For this review, use the dimensioned drawing (mm, ordinates from the lowest corner) and the shaded views. Coordinates: 2 decimals unless noted, no trailing zeros. Loops run counter-clockwise (first coordinate to the right, second up) from the corner with the lowest first, then second, coordinate; pieces in that order, holes last. Notation, with made-up numbers: (-8.5, -10.75) - (44.5, -10.75) arc R19 cw to (44.5, 26.25) - close; hole circle Ø4 at (33, 1). An arc over 180 degrees is marked (long way). Answer in a Markdown table with one row per item. Add a question column.
(1) For P1, Ø1.5, axis at x = 14, z = 13.5, coming from the -Y side; P2, Ø12, axis at y = 10.5, z = 23, coming from the -X side (1 decimal); P3, Ø9.5, axis at x = 20.93, z = 18, coming from the +Y side; P4, Ø3, axis at x = 24, y = 11, coming from the +Z side, all flat-tipped, find the tip position at first contact; note any pin that passes through.
(2) We need section C-C on x = 23.5. Write out the cut boundary in (y, z) (1 decimal).
(3) For line 1 along X through (y, z) = (18.25, 18); line 2 along Z through (x, y) = (14.75, 13.25) (1 decimal); line 3 along X through (y, z) = (6.75, 14), list the stretches that pass through material, from the lowest coordinate up.
(4) Mouldability with a two-part tool opening along X and no side actions: class the marked faces 1, 2 and 3 as +X half, -X half, draft (parallel to the pull), parting line (faces both ways), or undercut.
(5) We need section A-A on x = 14. Write out the cut boundary in (y, z), plus the area to 3 significant figures.
(6) We need section B-B on z = 6. Write out the cut boundary in (x, y).
(7) We need section D-D on z = 18. Write out the cut boundary in (x, y), plus the area to 3 significant figures.
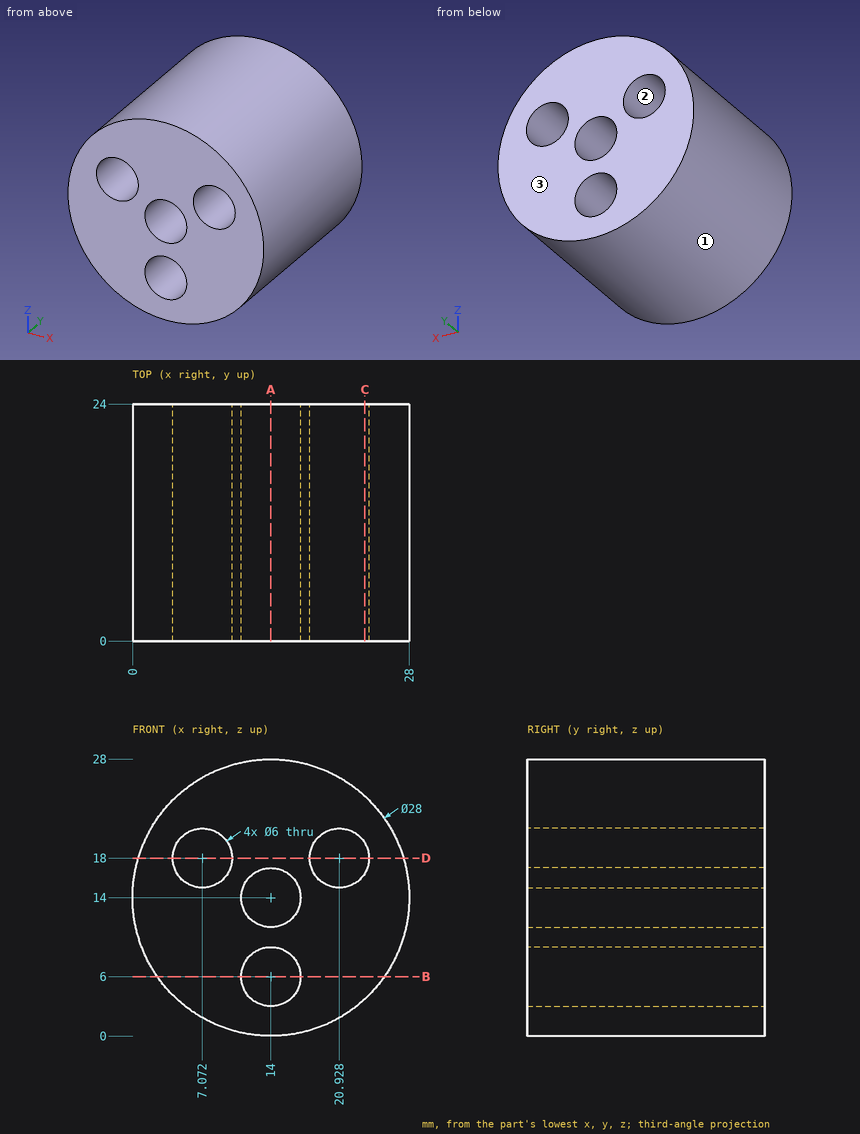
Outcome:
| question | item | result |
|---|---|---|
| 1 | P1 | through |
| 1 | P2 | x = 0.3 |
| 1 | P3 | y = 24 |
| 1 | P4 | z = 25.12 |
| 2 | outline | (0, 3.7) - (24, 3.7) - (24, 16.5) - (0, 16.5) - close; (0, 19.5) - (24, 19.5) - (24, 24.3) - (0, 24.3) - close |
| 3 | line 1 | 0.58 to 4.07, 10.07 to 17.93, 23.93 to 27.42 |
| 3 | line 2 | 0 to 3.1, 8.9 to 11.1, 16.9 to 28 |
| 3 | line 3 | 0 to 11, 17 to 28 |
| 4 | face 1 | parting line |
| 4 | face 2 | undercut |
| 4 | face 3 | draft |
| 5 | outline | (0, 0) - (24, 0) - (24, 3) - (0, 3) - close; (0, 9) - (24, 9) - (24, 11) - (0, 11) - close; (0, 17) - (24, 17) - (24, 28) - (0, 28) - close |
| 5 | area | 384 mm² |
| 6 | outline | (2.51, 0) - (11, 0) - (11, 24) - (2.51, 24) - close; (17, 0) - (25.49, 0) - (25.49, 24) - (17, 24) - close |
| 7 | outline | (0.58, 0) - (4.07, 0) - (4.07, 24) - (0.58, 24) - close; (10.07, 0) - (17.93, 0) - (17.93, 24) - (10.07, 24) - close; (23.93, 0) - (27.42, 0) - (27.42, 24) - (23.93, 24) - close |
| 7 | area | 356 mm² |
